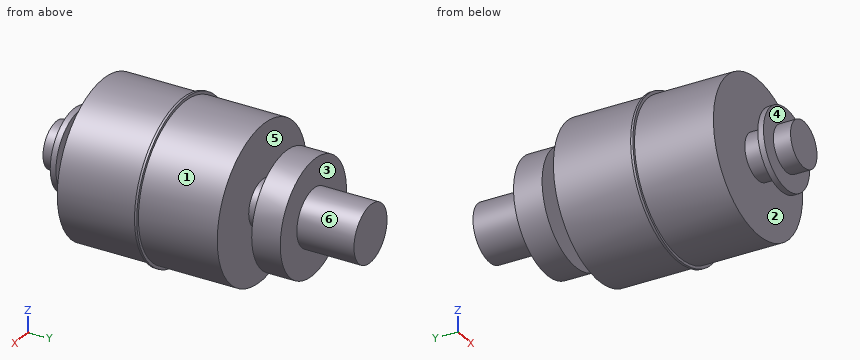
from build123d import *


with BuildPart() as part:
    # Sketch1 → Revolve1 (revolve)
    with BuildSketch(Plane.XY, mode=Mode.PRIVATE) as revolve1_sk:
        Polygon((0, 0), (0, 55), (-5, 55), (-5, 45), (-10, 45), (-10, 40), (-4, 40), (-4, 36), (-13.5, 36), (-13.5, 22.2), (-14, 22.2), (-14, 21.8), (-13.5, 21.8), (-13.5, 8), (-4, 8), (-4, 4), (-7, 4), (-7, 3), (-4, 3), (-4, 0), align=None)
    revolve(revolve1_sk.sketch.rotate(Axis((0, 0, 0), (0, 1, 0)), 180), axis=Axis((0, 0, 0), (0, 1, 0)))


solid = part.part
Can you work these out from the model? Positions are in its coordinate system, mm. Face numbers are marked on the shaded views. A direction names the side the tool comes from. Give positions to 0.01 mm unless a question says otherwise; leave off trailing zeros. Order: outer loops, then holes, each group sorted by start corner. A loop starts at its lowest first (then second) coordinate and runs counter-clockwise, first axis right, second up. Notation, with made-up numbers: M -29,87 L 12,87 A30 ccw 12,119 Z; hole C 36,77.5 d10. An arc over 180 degrees is marked long. Use a Markdown table: item, result. Add a question column.
Item 1: Suppose I cut it at D-D (y = 47.5). List the corners of the cut face in (x, z) for me.
Item 2: If I drill on L1, parallel to Y at x = 2.25, z = 4.75; L2, parallel to Y at x = -4.25, z = -7; L3, parallel to Y at x = 5, z = -12, over which ranges is the centre line in solid material (lowest first)? Write a range as [from, to].
Item 3: Suppose I cut it at B-B (y = 15). List the corners of the cut face in (x, z) for me, then the cut area to 3 significant figures.
Item 4: We'd pull the mould along Y, two halves only. Please class the marked faces 1, 2 and 3: +Y half, -Y half, draft (parallel to the pull), parting line (faces both ways), or undercut.
Item 5: For the marked faces 4, 5 and 6, which set-ups out of +Z, -Z, +X, -X, +Y, -Y let a thin tool reach every point of the face, with its end or its side?
Item 6: Suppose I cut it at A-A (x = 8.75). List the corners of the cut face in (y, z) for me, then the cut area to 3 significant figures.
Item 7: Suppose I cut it at C-C (x = -9.25). List the corners of the cut face in (y, z) for me.
Item 8: Will these pins go through, and if not, where does the flat tip stop? pin 1 (3 mm diameter, centred on y = 22, z = -3.5, fed in from -X); pin 2 (5 mm diameter, centred on y = 14.5, z = 0.5, fed in from -X); pin 3 (5 mm diameter, centred on x = -6.5, z = -11, fed in from -Y).
Answer sheet:
| question | item | result |
|---|---|---|
| 1 | outline | C 0,0 d10 |
| 2 | L1 | y = [3, 4], [8, 36], [40, 45] |
| 2 | L2 | y = [8, 36], [40, 45] |
| 2 | L3 | y = [8, 36] |
| 3 | outline | C 0,0 d27 |
| 3 | area | 573 mm² |
| 4 | face 1 | draft |
| 4 | face 2 | undercut |
| 4 | face 3 | +Y half |
| 5 | face 4 | -Y |
| 5 | face 5 | none |
| 5 | face 6 | +Y |
| 6 | outline | M 8,-10.28 L 21.8,-10.28 L 21.8,-10.93 L 22.2,-10.93 L 22.2,-10.28 L 36,-10.28 L 36,10.28 L 22.2,10.28 L 22.2,10.93 L 21.8,10.93 L 21.8,10.28 L 8,10.28 Z; M 40,-4.84 L 45,-4.84 L 45,4.84 L 40,4.84 Z |
| 6 | area | 625 mm² |
| 7 | outline | M 8,-9.83 L 21.8,-9.83 L 21.8,-10.51 L 22.2,-10.51 L 22.2,-9.83 L 36,-9.83 L 36,9.83 L 22.2,9.83 L 22.2,10.51 L 21.8,10.51 L 21.8,9.83 L 8,9.83 Z; M 40,-3.8 L 45,-3.8 L 45,3.8 L 40,3.8 Z |
| 8 | pin 1 | stops at x = -13.86 |
| 8 | pin 2 | stops at x = -13.5 |
| 8 | pin 3 | stops at y = 8 |
